```python
from build123d import *

# Parameters (mm, degrees)
SKETCH1_W           = 100
SKETCH1_H           = 100
BOSS_EXTRUDE1_DEPTH = 14
SKETCH2_R           = 25
CUT_EXTRUDE1_DEPTH  = 143.112631388
M8_TAPPED_HOLE1_D   = 6.8
FILLET1_R           = 10


with BuildPart() as part:
    # Sketch1 → Boss-Extrude1 (new body)
    with BuildSketch(Plane.XY):
        with Locations((50, -50)):
            Rectangle(SKETCH1_W, SKETCH1_H)
    extrude(amount=BOSS_EXTRUDE1_DEPTH)

    # Sketch2 → Cut-Extrude1 (cut, through all)
    with BuildSketch(Plane.XY.offset(14)):
        with Locations((50, -50)):
            Circle(SKETCH2_R)
    extrude(amount=-CUT_EXTRUDE1_DEPTH, mode=Mode.SUBTRACT)

    # M8 Tapped Hole1 (through all)
    with Locations(Plane.XY.offset(14)):
        with Locations((10, -10), (90, -10), (10, -90), (90, -90)):
            Hole(M8_TAPPED_HOLE1_D / 2)

    # Fillet1
    fillet1_edges = [part.edges().sort_by_distance(p)[0] for p in [
        (0, 0, 7),
        (100, 0, 7),
        (100, -100, 7),
        (0, -100, 7),
    ]]
    fillet(fillet1_edges, radius=FILLET1_R)


solid = part.part
```
Design review of the part built by this model. Coordinates are the model's own, in mm. Round coordinates to 2 decimals unless told otherwise and drop trailing zeros. Order: outer loops, then holes, each group sorted by start corner. A loop starts at its lowest first (then second) coordinate and runs counter-clockwise, first axis right, second up. Notation, with made-up numbers: M -30.75,-16 L 0.25,-16 A18 cw 0.25,-11 Z; hole C 16.25,50 d1. An arc over 180 degrees is marked long. Put each result on its own line as item: value.
Q1. Consider section C-C (z = 2). State the section outline as (x, y) points.
Reported:
outline: M 0,-90 A10 ccw 10,-100 L 90,-100 A10 ccw 100,-90 L 100,-10 A10 ccw 90,0 L 10,0 A10 ccw 0,-10 Z; hole C 10,-90 d6.8; hole C 10,-10 d6.8; hole C 50,-50 d50; hole C 90,-90 d6.8; hole C 90,-10 d6.8
Q2. Consider section B-B (y = -50). State the section outline as (x, z) points, and give its area (3 significant figures).
Reported:
outline: M 0,0 L 25,0 L 25,14 L 0,14 Z; M 75,0 L 100,0 L 100,14 L 75,14 Z
area: 700 mm²
Q3. Consider section D-D (x = 11.5). State the section outline as (y, z) points.
Reported:
outline: M -100,0 L -93.05,0 L -93.05,14 L -100,14 Z; M -86.95,0 L -13.05,0 L -13.05,14 L -86.95,14 Z; M -6.95,0 L 0,0 L 0,14 L -6.95,14 Z
Q4. To check wall thickness, follow line 1 (Y direction, x = 10, z = 7.25); line 2 (X direction, y = -51, z = 7.5); line 3 (Y direction, x = 51, z = 7.5). State the ranges of each line that lie inside material, in increasing order.
Reported:
line 1: -100 to -93.4, -86.6 to -13.4, -6.6 to 0
line 2: 0 to 25.02, 74.98 to 100
line 3: -100 to -74.98, -25.02 to 0
Q5. Draft analysis for pull direction Y (two halves, no side actions). For faces 1 (the face through (10.74, -93.32, 6.9)), 2 (the face through (49, 0, 7)), 3 (the face through (0, -51, 7)), 4 (the face through (93.4, -9.9, 6.9)), state which applies: released by +Y, released by -Y, zero draft, split by the parting line, or undercut.
Reported:
face 1: undercut
face 2: released by +Y
face 3: zero draft
face 4: undercut
Q6. Consider section A-A (x = 50). State the section outline as (y, z) points, and give its area (3 significant figures).
Reported:
outline: M -100,0 L -75,0 L -75,14 L -100,14 Z; M -25,0 L 0,0 L 0,14 L -25,14 Z
area: 700 mm²
Q7. Insertion check: pin 1 Ø8 at (x, y) = (68, -10) entering from -Z. The pin has a flat end and moves straight along its axis. Give the tip position at first contact, or say it passes through.
Reported:
pin 1: z = 0
